Geometry: see drawing. Coordinates: mm, zero at the bounding-box minimum. A direction names the side the tool comes from. Give positions to 0.01 mm unless a question says otherwise; leave off trailing zeros. Write each loop counter-clockwise with the first axis right and the second up, starting at its lowest first coordinate (ties: lowest second). Pieces come first, ordered by that corner, then holes. Notation, with made-up numbers: (48.25, -17) - (90.25, -17) arc R22 ccw to (90.25, 21) - close; hole circle Ø7 at (76.25, 43). An arc over 180 degrees is marked (long way). One line per question, with ' | ' between items. Start each with the question number.
(1) Ray query, line 1 (Z direction, x = 4, y = 7); line 2 (Z direction, x = 6, y = 4.5); line 3 (Z direction, x = 6.75, y = 10.5). Return the intervals inside material, ascending. Write a range as [from, to].
(2) Access query for the marked faces 1, 2 and 3. Directions: +Z, -Z, +X, -X, +Y, -Y. A direction counts if a zero-diameter tool reaches every point of the face in a straight line with its end or side. Return the directions, or none.
(3) Pin query (flat end, axial travel): pin 1 (2 mm diameter, centred on y = 8.5, z = 6, fed in from -X); pin 2 (3 mm diameter, centred on x = 9, y = 2.5, fed in from +Z); pin 3 (3 mm diameter, centred on y = 5, z = 7, fed in from -X). Return the tip coordinate at first contact, or that it passes through.
(4) Section C-C, the plane z = 11.5. Return loops of the section in (x, y).
(5) Section A-A, the plane y = 6.5. Return loops of the section in (x, z), plus the area to 3 significant figures.
(6) Section D-D, the plane z = 2. Return loops of the section in (x, y), plus the area to 3 significant figures.
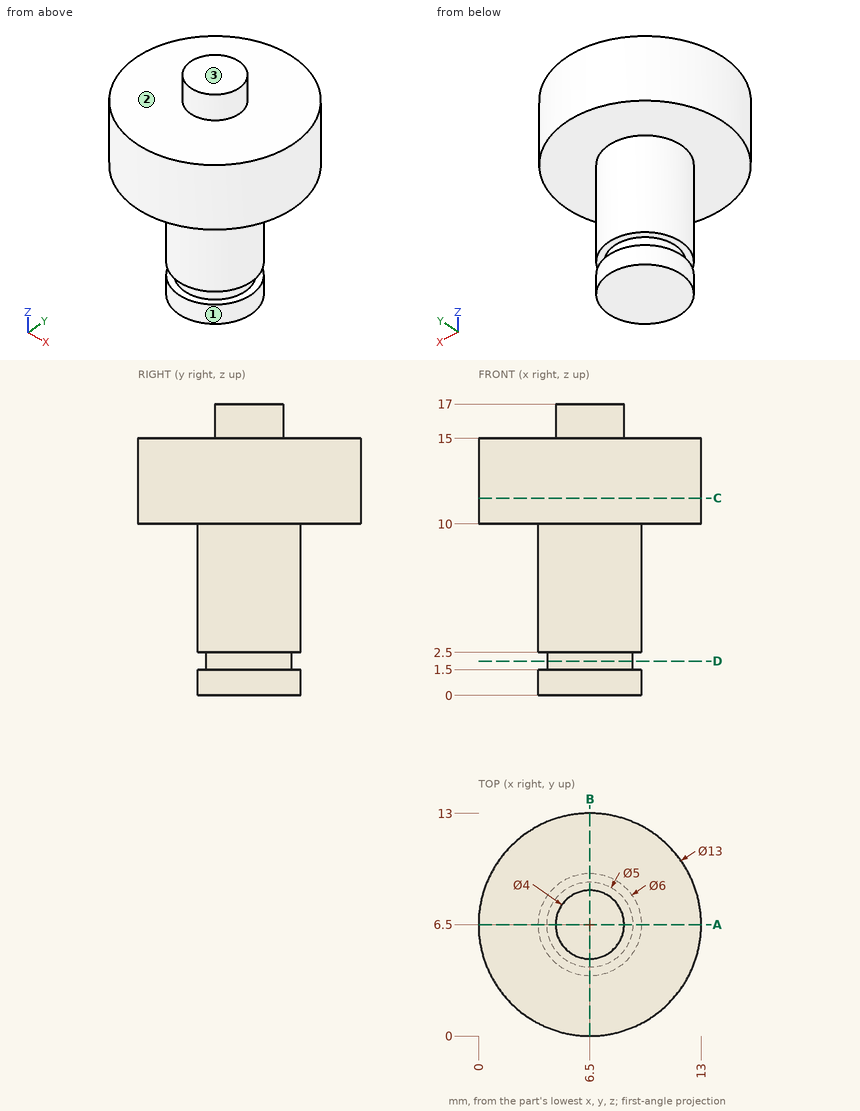
Check sheet entries:
1) line 1: [0, 1.5], [2.5, 15] | line 2: [0, 15] | line 3: [10, 15]
2) face 1: -Z | face 2: +Z | face 3: +Z, +X, -X, +Y, -Y
3) pin 1: x = 3.67 | pin 2: z = 15 | pin 3: x = 3.5
4) outline: circle Ø13 at (6.5, 6.5)
5) outline: (0, 10) - (3.5, 10) - (3.5, 2.5) - (4, 2.5) - (4, 1.5) - (3.5, 1.5) - (3.5, 0) - (9.5, 0) - (9.5, 1.5) - (9, 1.5) - (9, 2.5) - (9.5, 2.5) - (9.5, 10) - (13, 10) - (13, 15) - (8.5, 15) - (8.5, 17) - (4.5, 17) - (4.5, 15) - (0, 15) - close | area: 132 mm²
6) outline: circle Ø5 at (6.5, 6.5) | area: 19.6 mm²
